Check sheet for the modelled part. Datum: model origin and axes. Units: mm. A direction names the side the tool comes from. Round coordinates to 2 decimals unless told otherwise and drop trailing zeros. Write each loop counter-clockwise with the first axis right and the second up, starting at its lowest first coordinate (ties: lowest second). Pieces come first, ordered by that corner, then holes. Notation, with made-up numbers: (19, 58) -> (76, 58) arc R30 cw to (76, 92) -> close; hole circle Ø9 at (43, -26.5). An arc over 180 degrees is marked (long way). Use one line per item in the form item = value. Start each with the question number.
```python
from build123d import *

# Parameters (mm, degrees)
SKETCH1_R           = 12.5
SKETCH1_R_2         = 3.25
BOSS_EXTRUDE1_DEPTH = 59


with BuildPart() as part:
    # Sketch1 → Boss-Extrude1 (new, symmetric)
    with BuildSketch(Plane.XY):
        Circle(SKETCH1_R)
        Circle(SKETCH1_R_2, mode=Mode.SUBTRACT)
    extrude(amount=BOSS_EXTRUDE1_DEPTH, both=True)

    # Sketch3 → Cut-Revolve1 (revolve, cut)
    with BuildSketch(Plane(origin=(0, 0, 0), x_dir=(1, 0, 0), z_dir=(0, 1, 0))):
        Polygon((12.5, -50), (12.5, 50), (9.5, 38.803847577), (9.5, -38.803847577), align=None)
    revolve(axis=Axis((0, 0, 0), (0, 0, -1)), mode=Mode.SUBTRACT)


solid = part.part
```
1. Depth check by flat-ended pin: pin 1 (10 mm diameter, centred on x = 2.5, z = -14.5, fed in from +Y); pin 2 (12 mm diameter, centred on x = 9.5, z = -2.5, fed in from +Y); pin 3 (6 mm diameter, centred on x = 10, z = 16, fed in from +Y). Enter the tip coordinate at first touch or a pass-through.
2. Scan lines: probe 1 along Y at (x, z) = (0, -15); probe 2 along X at (y, z) = (0.5, 16); probe 3 along Y at (x, z) = (1, 31). Record each from-to range of solid material in increasing order.
3. Sectioned sample at C-C (z = 12). Enter the section's corners in (x, y).
4. Mould release check, pull along Z, two halves, no side actions. Record for faces 3 (the face through (3, -3, 59)), 4 (the face through (-8.184, 6.275, -41.836)), 5 (the face through (3, -3, -59)), 6 (the face through (-2.579, -1.978, -0.826)): +Z half, -Z half, draft (parallel to the pull), parting line (faces both ways), or undercut.
5. Sectioned sample at A-A (y = 0). Enter the section's corners in (x, z).
6. Sectioned sample at D-D (z = -41). Enter the section's corners in (x, y), and give its area (3 significant figures).
7. Tool access check on faces 1 (the face through (4.38, 8.43, 0.54)), 2 (the face through (11.923, 3.755, 54.563)). Record the directions out of +Z, -Z, +X, -X, +Y, -Y that give a thin tool (end or side, any length) a straight path to the whole face; none if there is none.
Returned:
q1.pin_1 = 9.5
q1.pin_2 = 8.83
q1.pin_3 = 6.42
q2.probe_1 = -9.5 to -3.25, 3.25 to 9.5
q2.probe_2 = -9.49 to -3.21, 3.21 to 9.49
q2.probe_3 = -9.45 to -3.09, 3.09 to 9.45
q3.outline = circle Ø19 at (0, 0); hole circle Ø6.5 at (0, 0)
q4.face_3 = +Z half
q4.face_4 = undercut
q4.face_5 = -Z half
q4.face_6 = draft
q5.outline = (-12.5, -59) -> (-3.25, -59) -> (-3.25, 59) -> (-12.5, 59) -> (-12.5, 50) -> (-9.5, 38.8) -> (-9.5, -38.8) -> (-12.5, -50) -> close; (3.25, -59) -> (12.5, -59) -> (12.5, -50) -> (9.5, -38.8) -> (9.5, 38.8) -> (12.5, 50) -> (12.5, 59) -> (3.25, 59) -> close
q6.outline = circle Ø20.18 at (0, 0); hole circle Ø6.5 at (0, 0)
q6.area = 287 mm^2
q7.face_1 = none
q7.face_2 = +Z, -Z
